Geometry: final body of the model. Coordinates: model frame, mm. Give positions to 0.01 mm unless a question says otherwise; leave off trailing zeros. Write each loop counter-clockwise with the first axis right and the second up, starting at its lowest first coordinate (ties: lowest second). Pieces come first, ordered by that corner, then holes.
Q1. Section A-A (z = -549.5). Return the cut outline in (x, y).
Q2. Line query: line 1 (Z direction, x = 766, y = 0.3); line 2 (X direction, y = 0.95, z = -357.5). Output: solid intervals per line, ascending.
Q3. Section C-C (x = 45). Return the cut outline in (y, z).
Q4. Section B-B (y = 0.35). Return the cut outline in (x, z), plus the area to 3 significant figures.
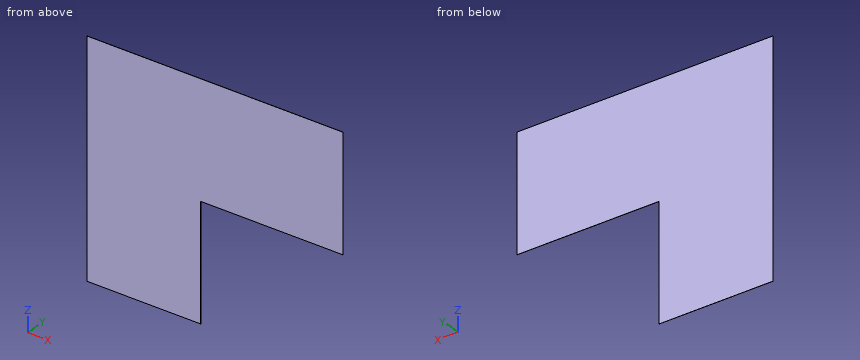
from build123d import *

# Parameters (mm, degrees)
BOSS_EXTRUDE1_DEPTH = 1


with BuildPart() as part:
    # Sketch1 → Boss-Extrude1 (new body)
    with BuildSketch(Plane(origin=(0, 0, 0), x_dir=(1, 0, 0), z_dir=(0, 1, 0))):
        Polygon((-900, -800), (900, -800), (900, 0), (0, 0), (-100, 0), (-100, 800), (-900, 800), align=None)
    extrude(amount=BOSS_EXTRUDE1_DEPTH)


solid = part.part
Computed:
1. outline: (-900, 0) - (-100, 0) - (-100, 1) - (-900, 1) - close
2. line 1: z = 0 to 800
2. line 2: x = -900 to -100
3. outline: (0, 0) - (1, 0) - (1, 800) - (0, 800) - close
4. outline: (-900, -800) - (-100, -800) - (-100, 0) - (900, 0) - (900, 800) - (-900, 800) - close
4. area: 2,080,000 mm2
